The listing builds one solid part. Answer for the finished solid, in the listing's coordinates (mm). Coordinates: 2 decimals unless noted, no trailing zeros. Order: outer loops, then holes, each group sorted by start corner. A loop starts at its lowest first (then second) coordinate and runs counter-clockwise, first axis right, second up. Notation, with made-up numbers: (26, 78.25) -> (64, 78.25) arc R13 ccw to (64, 88.25) -> close; hole circle Ø9 at (63.5, 27). An arc over 180 degrees is marked (long way). One line per question, with ' | ' between items.
from build123d import *

# Parameters (mm, degrees)
SKETCH1_R           = 15
SKETCH1_R_2         = 9.9
BOSS_EXTRUDE1_DEPTH = 5
SKETCH2_R           = 12
SKETCH2_R_2         = 9.9
BOSS_EXTRUDE2_DEPTH = 15
CHAMFER1_SIZE       = 1


with BuildPart() as part:
    # Sketch1 → Boss-Extrude1 (new body)
    with BuildSketch(Plane.XY):
        Circle(SKETCH1_R)
        Circle(SKETCH1_R_2, mode=Mode.SUBTRACT)
    extrude(amount=BOSS_EXTRUDE1_DEPTH)

    # Sketch2 → Boss-Extrude2 (add)
    with BuildSketch(Plane.XY.offset(5)):
        Circle(SKETCH2_R)
        Circle(SKETCH2_R_2, mode=Mode.SUBTRACT)
    extrude(amount=BOSS_EXTRUDE2_DEPTH)

    # Chamfer1
    chamfer1_edges = [part.edges().sort_by_distance(p)[0] for p in [
        (-12, 0, 20),
        (-9.9, 0, 20),
        (-15, 0, 0),
    ]]
    chamfer(chamfer1_edges, length=CHAMFER1_SIZE)


solid = part.part
Item 1: Find the intervals of material crossed by L1, parallel to Y at x = 0, z = 6.5; L2, parallel to Y at x = 3.5, z = 4.5, in increasing order.
Computed values:
L1: y = -12 to -9.9, 9.9 to 12 | L2: y = -14.59 to -9.26, 9.26 to 14.59
Item 2: Each of these flat-tipped pins is pushed along its axis until it touches: pin 1 Ø1 at (x, z) = (0.5, 13) entering from -Y; pin 2 Ø5 at (y, z) = (6.5, 3.5) entering from -X; pin 3 Ø12 at (x, z) = (5, 10) entering from +Y. Where does it stop, or does it pass through?
Computed values:
pin 1: stops at y = -12 | pin 2: stops at x = -14.46 | pin 3: stops at y = 14.91
Item 3: Determine the mould class of faces 1 (the face through (9.443, 2.974, 9.367)), 2 (the face through (-7, 10, 5)), 3 (the face through (-11.99, 0.53, 11.9)) for opening direction Y: pulls with the +Y half, pulls with the -Y half, needs draft (parallel to the pull), parting line crosses it, or undercut.
Computed values:
face 1: undercut | face 2: needs draft | face 3: parting line crosses it
Item 4: Section A-A, the plane y = 0 is taken. Give the vertices of the cut face in (x, z).
Computed values:
outline: (-15, 1) -> (-14, 0) -> (-9.9, 0) -> (-9.9, 19) -> (-10.9, 20) -> (-11, 20) -> (-12, 19) -> (-12, 5) -> (-15, 5) -> close; (9.9, 0) -> (14, 0) -> (15, 1) -> (15, 5) -> (12, 5) -> (12, 19) -> (11, 20) -> (10.9, 20) -> (9.9, 19) -> close
Item 5: Section C-C, the plane z = 11.75 is taken. Give the vertices of the cut face in (x, y), plus the area to 3 significant figures.
Computed values:
outline: circle Ø24 at (0, 0); hole circle Ø19.8 at (0, 0) | area: 144 mm^2
